from build123d import *
from build123d.topology import SkipClean

# Parameters (mm, degrees)
ARM_BODY_DEPTH            = 50
FRONT_LUG_SKETCH_R        = 30
FRONT_LUG_SKETCH_R_2      = 15
FRONT_LUG_30_DEPTH        = 15
REAR_START                = 15
REAR_LUG_SKETCH_R         = 30
REAR_LUG_SKETCH_R_2       = 15
REAR_LUG_30_DEPTH         = 15
TOP_SLOT_SKETCH_W         = 75
TOP_SLOT_SKETCH_H         = 20
TOP_SLOT_CUT_DEPTH        = 179.465683
LUG_RELIEF_CUT_DEPTH      = 173.771525
PIN_POST_SKETCH_R         = 15
PIN_POST_SKETCH_R_2       = 7.5
PIN_POST_15_DEPTH         = 40
SUPPORT_RIB_REACH         = 180.955
SUPPORT_RIB_SKETCH_WALL_W = 432.658256
SUPPORT_RIB_SKETCH_WALL_H = 20
EYE_BORE_SKETCH_R         = 15
EYE_BORE_DEPTH            = 187.145105


with BuildPart() as part:
    # Arm Profile Sketch → Arm Body (new body)
    with BuildSketch(Plane.XY):
        with BuildLine():
            Line((0, 0), (30, 0))
            Line((30, 0), (30, 40))
            Line((30, 40), (-10, 40))
            ThreePointArc((-10, 40), (-13.278154, 32.923449), (-21.022255, 32))
            Line((-21.022255, 32), (-155, 32))
            Line((-155, 32), (-155, -28))
            Line((-155, -28), (-60, -28))
            Line((-60, -28), (-60, 15))
            Line((-60, 15), (-8, 15))
            ThreePointArc((-8, 15), (-2.343146, 12.656854), (0, 7))
            Line((0, 7), (0, 0))
        make_face()
    extrude(amount=ARM_BODY_DEPTH)

    # Front Lug Sketch → Front Lug Ø30 (add)
    with BuildSketch(Plane.XY.offset(50)):
        with Locations(Location((-125, 2, 0), (0, 0, 180))):
            Circle(FRONT_LUG_SKETCH_R)
        with Locations((-125, 2)):
            Circle(FRONT_LUG_SKETCH_R_2, mode=Mode.SUBTRACT)
    extrude(amount=FRONT_LUG_30_DEPTH)

    # Rear Lug Sketch → Rear Lug Ø30 (add)
    with BuildSketch(Plane(origin=(0, 0, 0), x_dir=(-1, 0, 0), z_dir=(0, 0, -1)).offset(REAR_START)):
        with Locations((125, 2)):
            Circle(REAR_LUG_SKETCH_R)
        with Locations(Location((125, 2, 0), (0, 0, 180))):
            Circle(REAR_LUG_SKETCH_R_2, mode=Mode.SUBTRACT)
    extrude(amount=-REAR_LUG_30_DEPTH)

    # Top Slot Sketch → Top Slot Cut (cut, through all)
    with BuildSketch(Plane(origin=(0, 32, 0), x_dir=(1, 0, 0), z_dir=(0, 1, 0))):
        with Locations((-117.5, -25.955312)):
            Rectangle(TOP_SLOT_SKETCH_W, TOP_SLOT_SKETCH_H)
    extrude(amount=-TOP_SLOT_CUT_DEPTH, mode=Mode.SUBTRACT)

    # Lug Relief Sketch → Lug Relief Cut (cut, through all)
    with SkipClean():  # the faces are left unmerged after this step: merging them gives an invalid solid
        with BuildSketch(Plane.XY.offset(50)):
            with BuildLine():
                Line((-155, 32), (-125, 32))
                ThreePointArc((-125, 32), (-146.213203, 23.213203), (-155, 2))
                Line((-155, 2), (-155, 32))
            make_face()
        extrude(amount=-LUG_RELIEF_CUT_DEPTH, mode=Mode.SUBTRACT)

    # Pin Post Sketch → Pin Post Ø15 (add)
    with SkipClean():  # the faces are left unmerged after this step: merging them gives an invalid solid
        with BuildSketch(Plane(origin=(0, 40, 0), x_dir=(1, 0, 0), z_dir=(0, 1, 0))):
            with Locations(Location((10, -25, 0), (0, 0, 90))):
                Circle(PIN_POST_SKETCH_R)
            with Locations(Location((10, -25, 0), (0, 0, 270))):
                Circle(PIN_POST_SKETCH_R_2, mode=Mode.SUBTRACT)
        extrude(amount=PIN_POST_15_DEPTH)

    # Support Rib Sketch wall → Support Rib (add, up to next)
    with BuildSketch(Plane(origin=(-36.077613, 50.900721, 25), x_dir=(-0.854394921364, -0.519624208778, 0), z_dir=(0.519624208778, -0.854394921364, 0)), mode=Mode.PRIVATE) as support_rib_sk1:
        Rectangle(SUPPORT_RIB_SKETCH_WALL_W, SUPPORT_RIB_SKETCH_WALL_H)
    support_rib_tool1 = extrude(support_rib_sk1.sketch, amount=SUPPORT_RIB_REACH, mode=Mode.PRIVATE) - part.part
    add(support_rib_tool1.solids().sort_by_distance((-36.077613, 50.900721, 25))[0])

    # Eye Bore Sketch → Eye Bore (cut, through all)
    with SkipClean():  # the faces are left unmerged after this step: merging them gives an invalid solid
        with BuildSketch(Plane.XY.offset(50)):
            with Locations((-125, 2)):
                Circle(EYE_BORE_SKETCH_R)
        extrude(amount=-EYE_BORE_DEPTH, mode=Mode.SUBTRACT)


solid = part.part
The model under review builds one solid part; all positions refer to its coordinate system, in mm. A direction names the side the tool comes from. Give positions to 0.01 mm unless a question says otherwise; leave off trailing zeros. Order: outer loops, then holes, each group sorted by start corner. A loop starts at its lowest first (then second) coordinate and runs counter-clockwise, first axis right, second up. Notation, with made-up numbers: (17.5, 51) -> (34.5, 51) arc R30 ccw to (34.5, 79) -> close; hole circle Ø2 at (75.25, -36.75). An arc over 180 degrees is marked (long way). Write item = value, one per line. Start each with the question number.
(1) Take a section at B-B (y = -5.5). Write out the cut boundary in (x, z).
(2) For L1, parallel to X at y = 2, z = 9; L2, parallel to Y at x = -125, z = 40; L3, parallel to Z at x = -141, y = -14, list the stretches that pass through material, from the lowest coordinate up. Write a range as from..to.
(3) Take a section at C-C (z = 6). Write out the cut boundary in (x, y), plus the area to 3 significant figures.
(4) For pin 1 Ø7.5 at (y, z) = (2.5, 23.5) entering from -X; pin 2 Ø6 at (x, z) = (-84, -2.5) entering from +Y; pin 3 Ø1.5 at (x, z) = (-19, 27) entering from -Y, all flat-tipped, find the tip position at first contact; note any pin that passes through.
(5) Take a section at D-D (x = 10). Write out the cut boundary in (y, z).
(6) Tool access review of faces 4 (the cylindrical face through (5.436, 59.72, 19.048)), 5 (the flat face through (0, 4, 25)), 6 (the flat face through (-109.7, 2.4, 15.955)), 7 (the flat face through (-131, -12, 65)): name each direction out of +Z, -Z, +X, -X, +Y, -Y from which nothing blocks a thin tool from reaching the whole face with its end or side.
(7) Take a section at A-A (x = -103). Write out the cut boundary in (y, z), plus the area to 3 significant figures.
(8) Draft analysis for pull direction X (two halves, no side actions). For faces 1 (the flat face through (-155, -13, 43)), 2 (the cylindrical face through (-13.19, 32.99, 42.4)), 3 (the cylindrical face through (24.643, 59.72, 28.252)), state which applies: +X half, -X half, draft (parallel to the pull), parting line (faces both ways), or undercut.
Returned:
q1.outline = (-155, 0) -> (-154.05, 0) -> (-154.05, -15) -> (-137.99, -15) -> (-137.99, 15.96) -> (-155, 15.96) -> close; (-155, 35.96) -> (-137.99, 35.96) -> (-137.99, 65) -> (-154.05, 65) -> (-154.05, 50) -> (-155, 50) -> close; (-112.01, -15) -> (-95.95, -15) -> (-95.95, 0) -> (-60, 0) -> (-60, 50) -> (-95.95, 50) -> (-95.95, 65) -> (-112.01, 65) -> (-112.01, 35.96) -> (-80, 35.96) -> (-80, 15.96) -> (-112.01, 15.96) -> close
q2.L1 = -155..-140, -110..-60, 0..30
q2.L2 = -28..-13, 17..32
q2.L3 = -15..15.96, 35.96..65
q3.outline = (-155, -28) -> (-60, -28) -> (-60, 15) -> (-8, 15) arc R8 cw to (0, 7) -> (0, 0) -> (30, 0) -> (30, 40) -> (-10, 40) arc R8 cw to (-21.02, 32) -> (-125, 32) arc R30 ccw to (-155, 2) -> close; hole circle Ø30 at (-125, 2)
q3.area = 7,120 mm²
q4.pin_1 = -80
q4.pin_2 = 32
q4.pin_3 = 15
q5.outline = (0, 0) -> (40, 0) -> (40, 10) -> (80, 10) -> (80, 17.5) -> (40, 17.5) -> (40, 32.5) -> (80, 32.5) -> (80, 40) -> (40, 40) -> (40, 50) -> (0, 50) -> close
q6.face_4 = +Y
q6.face_5 = +Z, -Z, -Y
q6.face_6 = -X, +Y, -Y
q6.face_7 = +Z, +X, -X, +Y, -Y
q7.outline = (-28, 0) -> (-18.4, 0) -> (-18.4, -15) -> (22.4, -15) -> (22.4, 0) -> (32, 0) -> (32, 15.96) -> (-28, 15.96) -> close; (-28, 35.96) -> (32, 35.96) -> (32, 50) -> (22.4, 50) -> (22.4, 65) -> (-18.4, 65) -> (-18.4, 50) -> (-28, 50) -> close
q7.area = 3,020 mm²
q8.face_1 = -X half
q8.face_2 = undercut
q8.face_3 = parting line
